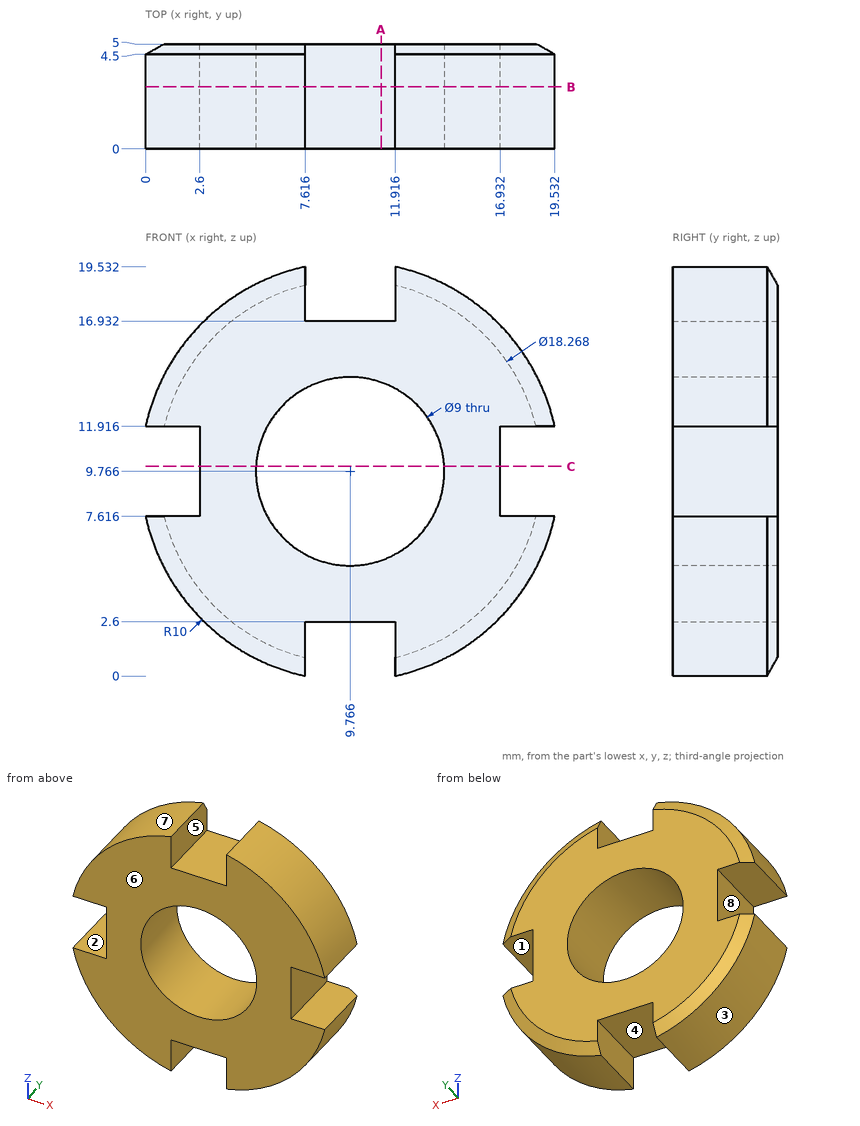
The drawing under review shows one solid part. Ordinate dimensions are in mm from its lowest x, y, z. A direction names the side the tool comes from. Coordinates: 2 decimals unless noted, no trailing zeros. Order: outer loops, then holes, each group sorted by start corner. A loop starts at its lowest first (then second) coordinate and runs counter-clockwise, first axis right, second up. Notation, with made-up numbers: M 10,57 L 42,57 A22 cw 42,65 Z; hole C 11.5,10 d4. An arc over 180 degrees is marked long. One line per question, with ' | ' between items.
(1) Machinability: for the marked faces 1, 2, 3, 4 and 5, which of the approach directions +Z, -Z, +X, -X, +Y, -Y give a long, thin tool a straight path to every point of the face, cutting with its end or side? Answer none if there is none.
Geometry results:
face 1: +X, +Y, -Y | face 2: -X, +Y, -Y | face 3: -Z, -X, +Y, -Y | face 4: -Z, +Y, -Y | face 5: +Z, +Y, -Y
(2) For probe 1 along Z at (x, y) = (10, 2.4); probe 2 along Z at (x, y) = (9, 0.65), list the stretches that pass through material, from the lowest coordinate up. Write a range as from..to.
Geometry results:
probe 1: z = 2.6..5.27, 14.26..16.93 | probe 2: z = 2.6..5.33, 14.2..16.93
(3) The part is to be moulded in two halves that separate along Z. For the marked faces 6, 7 and 8, say which applies: +Z half, -Z half, draft (parallel to the pull), parting line (faces both ways), or undercut.
Geometry results:
face 6: draft | face 7: +Z half | face 8: undercut
(4) Add section C-C, the plane z = 10. Write out the cut boundary in (x, y).
Geometry results:
outline: M 2.6,0 L 5.27,0 L 5.27,5 L 2.6,5 Z; M 14.26,0 L 16.93,0 L 16.93,5 L 14.26,5 Z
(5) Insertion check: pin 1 (2 mm diameter, centred on y = 2, z = 9.5, fed in from +X); pin 2 (1 mm diameter, centred on y = 2, z = 5.5, fed in from -X); pin 3 (3 mm diameter, centred on x = 18.5, y = 3, fed in from -Z). Each pin has a flat end and moves straight along its axis. Give the tip position at first contact, or say it passes through.
Geometry results:
pin 1: stops at x = 16.93 | pin 2: stops at x = 0.5 | pin 3: stops at z = 2.86
(6) Add section B-B, the plane y = 2.95. Write out the cut boundary in (x, z).
Geometry results:
outline: M 0,7.62 A10 ccw 7.62,0 L 7.62,2.6 L 11.92,2.6 L 11.92,0 A10 ccw 19.53,7.62 L 16.93,7.62 L 16.93,11.92 L 19.53,11.92 A10 ccw 11.92,19.53 L 11.92,16.93 L 7.62,16.93 L 7.62,19.53 A10 ccw 0,11.92 L 2.6,11.92 L 2.6,7.62 Z; hole C 9.77,9.77 d9
(7) Add section A-A, the plane x = 11.25. Write out the cut boundary in (y, z) (1 decimal), then the cut area to 3 significant figures.
Geometry results:
outline: M 0,2.6 L 5,2.6 L 5,5.5 L 0,5.5 Z; M 0,14 L 5,14 L 5,16.9 L 0,16.9 Z | area: 29.2 mm²
